Source: CAD feature listing. Evaluate the final solid. Frame: model axes, mm. Face numbers are marked on the shaded views. A direction names the side the tool comes from. Round coordinates to 2 decimals unless told otherwise and drop trailing zeros. Write each loop counter-clockwise with the first axis right and the second up, starting at its lowest first coordinate (ties: lowest second). Pieces come first, ordered by that corner, then holes. Notation, with made-up numbers: (51, 8.25) -> (69, 8.25) arc R20 cw to (69, 18.25) -> close; hole circle Ø11 at (34.25, 61.5). An arc over 180 degrees is marked (long way). Return JSON: item names as keys, results as strings. Group by question number.
from build123d import *

# Parameters (mm, degrees)
BASE_PLATE_SKETCH_W            = 9
BASE_PLATE_SKETCH_H            = 30
BASE_PLATE_DEPTH               = 9
LEFT_ARM_SKETCH_R              = 5.5
LEFT_ARM_DEPTH                 = 3
LEFT_ARM_UPRIGHT_DEPTH         = 9
LEFT_PIVOT_BOSS_SKETCH_R       = 10
LEFT_PIVOT_BOSS_SKETCH_R_2     = 5
LEFT_PIVOT_BOSS_20_DEPTH       = 31.5
LEFT_GUSSET_RIB_REACH          = 186.595
LEFT_GUSSET_SKETCH_WALL_W      = 403.142743776
LEFT_GUSSET_SKETCH_WALL_H      = 10
RIGHT_ARM_SKETCH_R             = 5.5
RIGHT_ARM_DEPTH                = 3
RIGHT_START                    = -9
RIGHT_ARM_UPRIGHT_DEPTH        = 9
RIGHT_PIVOT_BOSS_20_DEPTH      = 10
RIGHT_PIVOT_BOSS_20_DEPTH_BACK = 20
RIGHT_PIVOT_BOSS_SKETCH_R      = 10
RIGHT_PIVOT_BOSS_SKETCH_R_2    = 5
PIVOT_START                    = -38
PIVOT_CUT_SKETCH_R             = 5
PIVOT_CUT_DEPTH                = 38


with BuildPart() as part:
    # Base Plate Sketch → Base Plate (new, symmetric)
    with BuildSketch(Plane.XY):
        with BuildLine():
            Line((-7, 30), (7, 30))
            ThreePointArc((7, 30), (11.242640687, 28.242640687), (13, 24))
            Line((13, 24), (13, 0))
            Line((13, 0), (33, 0))
            Line((33, 0), (33, 89))
            Line((33, 89), (11, 89))
            Line((11, 89), (-3, 45))
            Line((-3, 45), (-33, 45))
            Line((-33, 45), (-33, 0))
            Line((-33, 0), (-13, 0))
            Line((-13, 0), (-13, 24))
            ThreePointArc((-13, 24), (-11.242640687, 28.242640687), (-7, 30))
        make_face()
        with Locations((19.5, 60)):
            Rectangle(BASE_PLATE_SKETCH_W, BASE_PLATE_SKETCH_H, mode=Mode.SUBTRACT)
    extrude(amount=BASE_PLATE_DEPTH, both=True)

    # Left Arm Sketch → Left Arm (add, symmetric)
    with BuildSketch(Plane.XY):
        with BuildLine():
            Line((33, 0), (61, 0))
            ThreePointArc((61, 0), (70.192388155, 3.807611845), (74, 13))
            Line((74, 13), (74, 80))
            Line((74, 80), (33, 80))
            Line((33, 80), (33, 0))
        make_face()
        with Locations((61, 13)):
            Circle(LEFT_ARM_SKETCH_R, mode=Mode.SUBTRACT)
    extrude(amount=LEFT_ARM_DEPTH, both=True)

    # Left Arm Upright Sketch → Left Arm Upright (add)
    with BuildSketch(Plane(origin=(74, 0, 0), x_dir=(0, 0, -1), z_dir=(1, 0, 0))):
        with BuildLine():
            Line((-12, 45), (12, 45))
            Line((12, 45), (12, 139))
            ThreePointArc((12, 139), (0, 151), (-12, 139))
            Line((-12, 139), (-12, 45))
        make_face()
    extrude(amount=-LEFT_ARM_UPRIGHT_DEPTH)

    # Left Pivot Boss Sketch → Left Pivot Boss Ø20 (add)
    with BuildSketch(Plane(origin=(74, 0, 0), x_dir=(0, 0, -1), z_dir=(1, 0, 0))):
        with Locations(Location((0, 139, 0), (0, 0, 180))):
            Circle(LEFT_PIVOT_BOSS_SKETCH_R)
        with Locations((0, 139)):
            Circle(LEFT_PIVOT_BOSS_SKETCH_R_2, mode=Mode.SUBTRACT)
    extrude(amount=LEFT_PIVOT_BOSS_20_DEPTH)

    # Left Gusset Sketch wall → Left Gusset Rib (add, up to next)
    with BuildSketch(Plane(origin=(79.5, 114, 0), x_dir=(-0.344254649158, -0.938876315887, 0), z_dir=(0.938876315887, -0.344254649158, 0)), mode=Mode.PRIVATE) as left_gusset_rib_sk1:
        Rectangle(LEFT_GUSSET_SKETCH_WALL_W, LEFT_GUSSET_SKETCH_WALL_H)
    left_gusset_rib_tool1 = extrude(left_gusset_rib_sk1.sketch, amount=-LEFT_GUSSET_RIB_REACH, mode=Mode.PRIVATE) - part.part
    add(left_gusset_rib_tool1.solids().sort_by_distance((79.5, 114, 0))[0])

    # Right Arm Sketch → Right Arm (add, symmetric)
    with BuildSketch(Plane.XY):
        with BuildLine():
            Line((-33, 0), (-57, 0))
            ThreePointArc((-57, 0), (-66.192388155, 3.807611845), (-70, 13))
            Line((-70, 13), (-70, 100))
            Line((-70, 100), (-50, 100))
            Line((-50, 100), (-33, 45))
            Line((-33, 45), (-33, 0))
        make_face()
        with Locations((-57, 13)):
            Circle(RIGHT_ARM_SKETCH_R, mode=Mode.SUBTRACT)
    extrude(amount=RIGHT_ARM_DEPTH, both=True)

    # Right Arm Upright Sketch → Right Arm Upright (add)
    with BuildSketch(Plane.ZY.offset(70).offset(RIGHT_START)):
        with BuildLine():
            Line((12, 45), (-12, 45))
            Line((-12, 45), (-12, 139))
            ThreePointArc((-12, 139), (0, 151), (12, 139))
            Line((12, 139), (12, 45))
        make_face()
    extrude(amount=RIGHT_ARM_UPRIGHT_DEPTH)

    # Right Pivot Boss Sketch → Right Pivot Boss Ø20 (add, two sides: drawn at the far end of the back side and taken through both)
    with BuildSketch(Plane.ZY.offset(70).offset(-RIGHT_PIVOT_BOSS_20_DEPTH_BACK)):
        with Locations(Location((0, 139, 0), (0, 0, 300))):
            Circle(RIGHT_PIVOT_BOSS_SKETCH_R)
        with Locations(Location((0, 139, 0), (0, 0, 180))):
            Circle(RIGHT_PIVOT_BOSS_SKETCH_R_2, mode=Mode.SUBTRACT)
    extrude(amount=RIGHT_PIVOT_BOSS_20_DEPTH + RIGHT_PIVOT_BOSS_20_DEPTH_BACK)

    # Pivot Cut Sketch → Pivot Cut (cut)
    with BuildSketch(Plane(origin=(-50, 0, 0), x_dir=(0, 0, -1), z_dir=(1, 0, 0)).offset(PIVOT_START)):
        with Locations((0, 139)):
            Circle(PIVOT_CUT_SKETCH_R)
    extrude(amount=PIVOT_CUT_DEPTH, mode=Mode.SUBTRACT)


solid = part.part
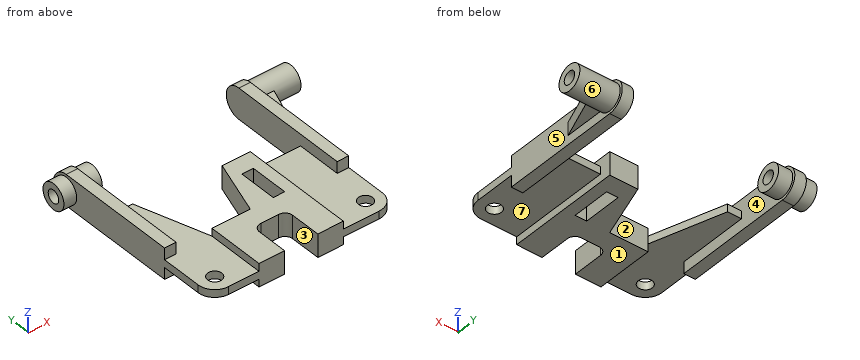
Item 1: Set-up query: the marked faces 1, 2, 3 and 4. Return all of +Z, -Z, +X, -X, +Y, -Y with unobstructed straight access to the full face (end or side cutting, diameter ignored); none if empty.
Item 2: Cut plane D-D on x = 57.5. Output: boundary loops of the cut face in (y, z).
Item 3: First-contact query: pin 1 Ø1 at (y, z) = (109.5, 6.5) entering from +X; pin 2 Ø10 at (x, z) = (17.5, 1.5) entering from +Y; pin 3 Ø5 at (y, z) = (32, -5) entering from -X; pin 4 Ø1.5 at (x, z) = (24.5, -5.5) entering from -Y. Flat tips, straight axial feed; report the tip coordinate or a pass-through.
Item 4: Pull-direction query (X, two-part tool) for the marked faces 5, 6 and 7; classes: +X half, -X half, draft (parallel to the pull), parting line (faces both ways), or undercut.
Item 5: Cut plane B-B on y = 63.5. Output: boundary loops of the cut face in (x, z).
Item 6: Material intervals for probe 1 along Y at (x, z) = (-57, 0.5); probe 2 along X at (y, z) = (115, 6.5); probe 3 along Y at (x, z) = (61, -1), sorted ascending.
Item 7: Cut plane A-A on y = 121.5. Output: boundary loops of the cut face in (x, z).
Item 8: Cut plane C-C on z = -1. Give the number of separate pieces and of enclosed holes in the cut face, and give its area (3 significant figures).
Here are the results:
{
 "1": {"face 1": "-Z, +Y, -Y", "face 2": "+Z, -Z, +Y", "face 3": "+Z, -Z, -Y", "face 4": "none"},
 "2": {"outline": "(0, -3) -> (8.76, -3) -> (8.76, 3) -> (0, 3) -> close; (17.24, -3) -> (80, -3) -> (80, 3) -> (17.24, 3) -> close"},
 "3": {"pin 1": "stops at x = 74", "pin 2": "stops at y = 89", "pin 3": "stops at x = -70", "pin 4": "stops at y = 0"},
 "4": {"face 5": "+X half", "face 6": "draft", "face 7": "undercut"},
 "5": {"outline": "(-70, -12) -> (-61, -12) -> (-61, -3) -> (-38.72, -3) -> (-38.72, 3) -> (-61, 3) -> (-61, 12) -> (-70, 12) -> close; (2.89, -9) -> (15, -9) -> (15, 9) -> (2.89, 9) -> close; (24, -9) -> (33, -9) -> (33, -3) -> (65, -3) -> (65, -12) -> (74, -12) -> (74, 12) -> (65, 12) -> (65, 3) -> (33, 3) -> (33, 9) -> (24, 9) -> close"},
 "6": {"probe 1": "y = 0 to 7.5, 18.5 to 100, 129.01 to 134.03, 143.97 to 148.99", "probe 2": "x = -70 to -61, 65 to 74", "probe 3": "y = 0 to 7.5, 18.5 to 80"},
 "7": {"outline": "(-70, -12) -> (-61, -12) -> (-61, 12) -> (-70, 12) -> close; (65, -12) -> (74, -12) -> (74, -5) -> (82.25, -5) -> (82.25, 5) -> (74, 5) -> (74, 12) -> (65, 12) -> close"},
 "8": {"separate pieces": "2", "enclosed holes": "3", "area": "11,200 mm^2"}
}
